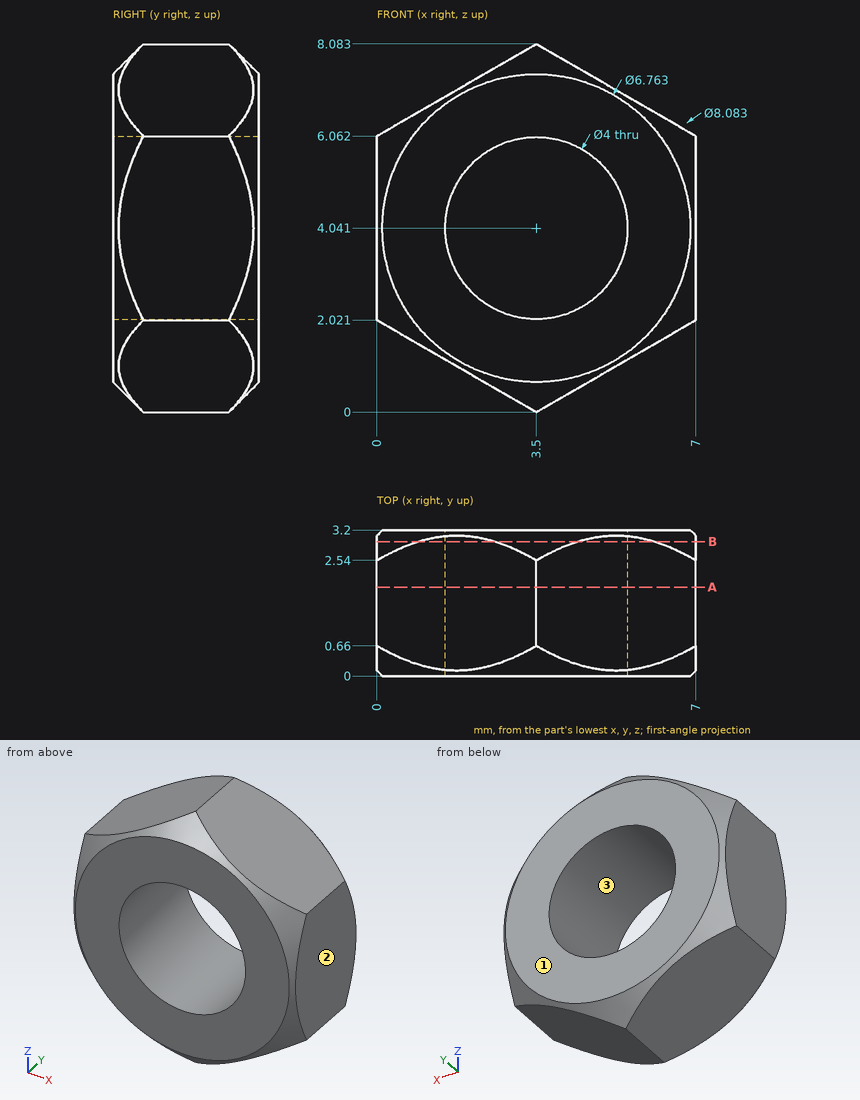
Input: dimensioned drawing with shaded views. Units: mm. Origin: part minimum x, y, z. Round coordinates to 2 decimals unless told otherwise and drop trailing zeros. Order: outer loops, then holes, each group sorted by start corner. A loop starts at its lowest first (then second) coordinate and runs counter-clockwise, first axis right, second up. Notation, with made-up numbers: (-24, 65.25) - (1, 65.25) arc R14 cw to (1, 75.25) - close; hole circle Ø1 at (8.5, -36). An arc over 180 degrees is marked (long way). Write item = value, one per line. Start each with the question number.
Q1. Ray query, line 1 (X direction, y = 0.8, z = 5.5); line 2 (X direction, y = 0.35, z = 3); line 3 (Z direction, x = 4, y = 2.35) (1 decimal). Return the intervals inside material, ascending. Write a range as from..to.
Q2. Cut plane B-B on y = 2.95. Return the cut outline in (x, z) (1 decimal).
Q3. Pin query (flat end, axial travel): pin 1 (3 mm diameter, centred on x = 1, z = 2.5, fed in from -Y). Return the tip coordinate at first contact, or that it passes through.
Q4. Cut plane A-A on y = 1.95. Return the cut outline in (x, z).
Q5. Pull-direction query (X, two-part tool) for the marked faces 1, 2 and 3; classes: +X half, -X half, draft (parallel to the pull), parting line (faces both ways), or undercut.
Outcome:
q1.line_1 = 0..2.13, 4.87..7
q1.line_2 = 0..1.79, 5.21..7
q1.line_3 = 0.3..2.1, 6..7.8
q2.outline = (0, 3.1) arc R3.6 ccw to (0.9, 1.5) - (2.6, 0.5) arc R3.6 ccw to (4.4, 0.5) - (6.1, 1.5) arc R3.6 ccw to (7, 3.1) - (7, 5) arc R3.6 ccw to (6.1, 6.6) - (4.4, 7.6) arc R3.6 ccw to (2.6, 7.6) - (0.9, 6.6) arc R3.6 ccw to (0, 5) - close; hole circle Ø4 at (3.5, 4)
q3.pin_1 = 0
q4.outline = (0, 2.02) - (3.5, 0) - (7, 2.02) - (7, 6.06) - (3.5, 8.08) - (0, 6.06) - close; hole circle Ø4 at (3.5, 4.04)
q5.face_1 = draft
q5.face_2 = +X half
q5.face_3 = undercut
